The listing builds one solid part. Answer for the finished solid, in the listing's coordinates (mm). Face numbers are marked on the shaded views. A direction names the side the tool comes from. Round coordinates to 2 decimals unless told otherwise and drop trailing zeros. Loops run counter-clockwise (first coordinate to the right, second up) from the corner with the lowest first, then second, coordinate; pieces in that order, holes last. Notation, with made-up numbers: (46, 21) -> (96, 21) arc R12 cw to (96, 39) -> close; hole circle Ø8 at (73, -37.75). An arc over 180 degrees is marked (long way). Use a Markdown table: item, result. Add a question column.
Q1. Section C-C on y = -3.75 is taken. Give the vertices of the cut face in (x, z).
Q2. Consider line 1 (X direction, y = -2.25, z = 0); line 2 (Y direction, x = 2, z = 12); line 3 (X direction, y = 7.75, z = 0). Determine where each line is inside the solid, lowest interval first.
Q3. Given pin 1 Ø10 at (x, y) = (9, 4.5) entering from +Z, flat-ended and moving along its own axis, determine where the tip first touches the part or whether it passes through.
Q4. Which of the six approach directions +Z, -Z, +X, -X, +Y, -Y give full straight-line access (tool end or side, diameter ignored) to the marked faces 4 and 5?
Q5. Section B-B on y = 4.75 is taken. Give the vertices of the cut face in (x, z), then the cut area to 3 significant figures.
Q6. For a pull along X with two mould halves and no side action, classify the marked faces 1, 2 and 3 as released by +X, released by -X, zero draft, split by the parting line, or undercut.
Q7. Section A-A on z = 0 is taken. Give the vertices of the cut face in (x, y).
from build123d import *

# Parameters (mm, degrees)
BOSS_EXTRUDE1_DEPTH = 10
SKETCH2_R           = 5
CUT_EXTRUDE1_DEPTH  = 50
CUT_EXTRUDE2_START  = -15
SKETCH3_R           = 14
CUT_EXTRUDE2_DEPTH  = 4


with BuildPart() as part:
    # Sketch1 → Boss-Extrude1 (new, symmetric)
    with BuildSketch(Plane(origin=(0, 0, 0), x_dir=(1, 0, 0), z_dir=(0, 1, 0))):
        Polygon((0, 18.475208614), (-16, 9.237604307), (-16, -9.237604307), (0, -18.475208614), (16, -9.237604307), (16, 9.237604307), align=None)
    extrude(amount=BOSS_EXTRUDE1_DEPTH, both=True)

    # Sketch2 → Cut-Extrude1 (cut)
    with BuildSketch(Plane(origin=(0, 10, 0), x_dir=(1, 0, 0), z_dir=(0, 1, 0))):
        with Locations(Location((0, 0, 0), (0, 0, 270))):
            Circle(SKETCH2_R)
    extrude(amount=-CUT_EXTRUDE1_DEPTH, mode=Mode.SUBTRACT)

    # Sketch3 → Cut-Extrude2 (cut)
    with BuildSketch(Plane(origin=(0, 10, 0), x_dir=(1, 0, 0), z_dir=(0, 1, 0)).offset(CUT_EXTRUDE2_START)):
        with Locations(Location((0, 0, 0), (0, 0, 270))):
            Circle(SKETCH3_R)
    extrude(amount=CUT_EXTRUDE2_DEPTH, mode=Mode.SUBTRACT)

    # Sketch4 → Cut-Revolve1 (revolve, cut)
    with BuildSketch(Plane(origin=(0, 0, 0), x_dir=(0, 0, -1), z_dir=(1, 0, 0))):
        Polygon((18.475208614, 7.416237102), (18.475208614, 10), (14, 10), align=None)
    cut_revolve1 = revolve(axis=Axis((0, 0, 0), (0, 1, 0)), mode=Mode.SUBTRACT)

    # Mirror1: Cut-Revolve1 across plane
    add(cut_revolve1.mirror(Plane.ZX), mode=Mode.SUBTRACT)


solid = part.part
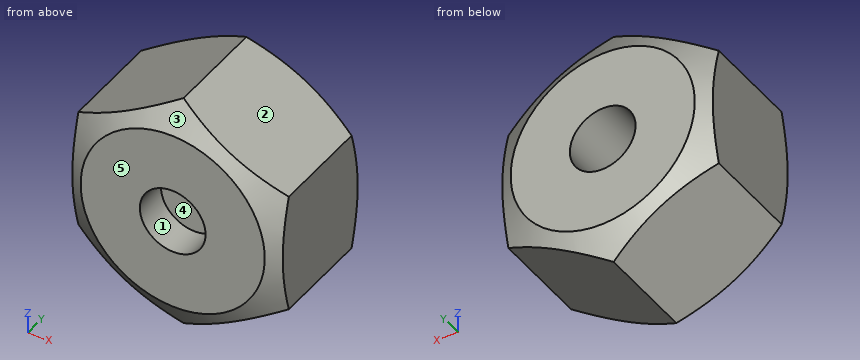
Checked values:
| question | item | result |
|---|---|---|
| 1 | outline | (-16, -9.24) -> (0, -18.48) -> (16, -9.24) -> (16, 9.24) -> (0, 18.48) -> (-16, 9.24) -> close; hole circle Ø28 at (0, 0) |
| 2 | line 1 | x = -16 to -14, 14 to 16 |
| 2 | line 2 | y = -10 to -5, -1 to 10 |
| 2 | line 3 | x = -16 to -5, 5 to 16 |
| 3 | pin 1 | stops at z = 16.17 |
| 4 | face 4 | none |
| 4 | face 5 | +Z, -Z, +X, -X, -Y |
| 5 | outline | (-16, -9.24) -> (0, -18.48) -> (16, -9.24) -> (16, 9.24) -> (0, 18.48) -> (-16, 9.24) -> close; hole circle Ø10 at (0, 0) |
| 5 | area | 808 mm2 |
| 6 | face 1 | undercut |
| 6 | face 2 | released by +X |
| 6 | face 3 | split by the parting line |
| 7 | outline | (-16, -8.85) -> (-14, -10) -> (-5, -10) -> (-5, -5) -> (-14, -5) -> (-14, -1) -> (-5, -1) -> (-5, 10) -> (-14, 10) -> (-16, 8.85) -> close; (5, -10) -> (14, -10) -> (16, -8.85) -> (16, 8.85) -> (14, 10) -> (5, 10) -> (5, -1) -> (14, -1) -> (14, -5) -> (5, -5) -> close |
